Verification items for the finished model (mm, model axes). A direction names the side the tool comes from. Give positions to 0.01 mm unless a question says otherwise; leave off trailing zeros. Loops run counter-clockwise (first coordinate to the right, second up) from the corner with the lowest first, then second, coordinate; pieces in that order, holes last. Notation, with made-up numbers: M 47.5,-37 L 79.5,-37 A21 cw 79.5,-26 Z; hole C 21.5,76.25 d5. An arc over 180 degrees is marked long. Write each question's results on one line, items separated by ' | '. Start each with the question number.
```python
from build123d import *

# Parameters (mm, degrees)
FRAME_BODY_DEPTH         = 40
FRAME_WINDOW_CUT_DEPTH   = 40
SIDE_LUG_A_DEPTH         = 13
SPIGOT_A_SKETCH_R        = 15
SPIGOT_A_SKETCH_R_2      = 7.5
SPIGOT_A_30_DEPTH        = 25
SIDE_START               = 13
SIDE_LUG_B_DEPTH         = 13
SPIGOT_START             = 25
SPIGOT_B_SKETCH_R        = 15
SPIGOT_B_SKETCH_R_2      = 7.5
SPIGOT_B_30_DEPTH        = 25
SPIGOT_EDGE_FILLETS_R2_R = 2
LUG_BLEND_FILLETS_R1_R   = 1


with BuildPart() as part:
    # Frame Profile Sketch → Frame Body (new body)
    with BuildSketch(Plane.XY):
        with BuildLine():
            Line((-12, -64), (12, -64))
            ThreePointArc((12, -64), (21.899494937, -59.899494937), (26, -50))
            Line((26, -50), (26, 50))
            ThreePointArc((26, 50), (21.899494937, 59.899494937), (12, 64))
            Line((12, 64), (-12, 64))
            ThreePointArc((-12, 64), (-21.899494937, 59.899494937), (-26, 50))
            Line((-26, 50), (-26, -50))
            ThreePointArc((-26, -50), (-21.899494937, -59.899494937), (-12, -64))
        make_face()
    extrude(amount=FRAME_BODY_DEPTH)

    # Frame Window Sketch → Frame Window Cut (cut)
    with BuildSketch(Plane.XY.offset(40)):
        with BuildLine():
            Line((14, -35), (14, 35))
            ThreePointArc((14, 35), (18.242640687, 36.757359313), (20, 41))
            Line((20, 41), (20, 50))
            ThreePointArc((20, 50), (18.242640687, 54.242640687), (14, 56))
            Line((14, 56), (-14, 56))
            ThreePointArc((-14, 56), (-18.242640687, 54.242640687), (-20, 50))
            Line((-20, 50), (-20, 41))
            ThreePointArc((-20, 41), (-18.242640687, 36.757359313), (-14, 35))
            Line((-14, 35), (-14, -35))
            ThreePointArc((-14, -35), (-18.242640687, -36.757359313), (-20, -41))
            Line((-20, -41), (-20, -50))
            ThreePointArc((-20, -50), (-18.242640687, -54.242640687), (-14, -56))
            Line((-14, -56), (14, -56))
            ThreePointArc((14, -56), (18.242640687, -54.242640687), (20, -50))
            Line((20, -50), (20, -41))
            ThreePointArc((20, -41), (18.242640687, -36.757359313), (14, -35))
        make_face()
    extrude(amount=-FRAME_WINDOW_CUT_DEPTH, mode=Mode.SUBTRACT)

    # Side Lug A Sketch → Side Lug A (add)
    with BuildSketch(Plane(origin=(26, 0, 0), x_dir=(0, 0, -1), z_dir=(1, 0, 0))):
        with BuildLine():
            Line((-40, 15), (-40, -15))
            ThreePointArc((-40, -15), (-37.914229564, -17.437900652), (-35.533410394, -19.588597743))
            ThreePointArc((-35.533410394, -19.588597743), (-29.708548536, -15.576576016), (-22.978505654, -17.751859172))
            ThreePointArc((-22.978505654, -17.751859172), (-20, -18), (-17.021494346, -17.751859172))
            ThreePointArc((-17.021494346, -17.751859172), (-10.291451464, -15.576576016), (-4.466589606, -19.588597743))
            ThreePointArc((-4.466589606, -19.588597743), (-2.085770436, -17.437900652), (0, -15))
            Line((0, -15), (0, 15))
            ThreePointArc((0, 15), (-2.085770436, 17.437900652), (-4.466589606, 19.588597743))
            ThreePointArc((-4.466589606, 19.588597743), (-10.291451464, 15.576576016), (-17.021494346, 17.751859172))
            ThreePointArc((-17.021494346, 17.751859172), (-20, 18), (-22.978505654, 17.751859172))
            ThreePointArc((-22.978505654, 17.751859172), (-29.708548536, 15.576576016), (-35.533410394, 19.588597743))
            ThreePointArc((-35.533410394, 19.588597743), (-37.914229564, 17.437900652), (-40, 15))
        make_face()
    extrude(amount=SIDE_LUG_A_DEPTH)

    # Spigot A Sketch → Spigot A Ø30 (add)
    with BuildSketch(Plane(origin=(39, 0, 0), x_dir=(0, 0, -1), z_dir=(1, 0, 0))):
        with Locations((-20, 0)):
            Circle(SPIGOT_A_SKETCH_R)
        with Locations((-20, 0)):
            Circle(SPIGOT_A_SKETCH_R_2, mode=Mode.SUBTRACT)
    extrude(amount=SPIGOT_A_30_DEPTH)

    # Side Lug B Sketch → Side Lug B (add)
    with BuildSketch(Plane.ZY.offset(26).offset(SIDE_START)):
        with BuildLine():
            Line((0, 15), (0, -15))
            ThreePointArc((0, -15), (2.085770436, -17.437900652), (4.466589606, -19.588597743))
            ThreePointArc((4.466589606, -19.588597743), (10.291451464, -15.576576016), (17.021494346, -17.751859172))
            ThreePointArc((17.021494346, -17.751859172), (20, -18), (22.978505654, -17.751859172))
            ThreePointArc((22.978505654, -17.751859172), (29.708548536, -15.576576016), (35.533410394, -19.588597743))
            ThreePointArc((35.533410394, -19.588597743), (37.914229564, -17.437900652), (40, -15))
            Line((40, -15), (40, 15))
            ThreePointArc((40, 15), (37.914229564, 17.437900652), (35.533410394, 19.588597743))
            ThreePointArc((35.533410394, 19.588597743), (29.708548536, 15.576576016), (22.978505654, 17.751859172))
            ThreePointArc((22.978505654, 17.751859172), (20, 18), (17.021494346, 17.751859172))
            ThreePointArc((17.021494346, 17.751859172), (10.291451464, 15.576576016), (4.466589606, 19.588597743))
            ThreePointArc((4.466589606, 19.588597743), (2.085770436, 17.437900652), (0, 15))
        make_face()
    extrude(amount=-SIDE_LUG_B_DEPTH)

    # Spigot B Sketch → Spigot B Ø30 (add)
    with BuildSketch(Plane.ZY.offset(39).offset(SPIGOT_START)):
        with Locations(Location((20, 0, 0), (0, 0, 180))):
            Circle(SPIGOT_B_SKETCH_R)
        with Locations(Location((20, 0, 0), (0, 0, 180))):
            Circle(SPIGOT_B_SKETCH_R_2, mode=Mode.SUBTRACT)
    extrude(amount=-SPIGOT_B_30_DEPTH)

    # Spigot Edge Fillets R2
    spigot_edge_fillets_r2_edges = [part.edges().sort_by_distance(p)[0] for p in [
        (64, 0, 35),
        (-64, 0, 35),
    ]]
    fillet(spigot_edge_fillets_r2_edges, radius=SPIGOT_EDGE_FILLETS_R2_R)

    # Lug Blend Fillets R1
    lug_blend_fillets_r1_edges = [part.edges().sort_by_distance(p)[0] for p in [
        (39, 0, 35),
        (-39, 0, 35),
    ]]
    fillet(lug_blend_fillets_r1_edges, radius=LUG_BLEND_FILLETS_R1_R)


solid = part.part
```
1. Thickness scan on probe 1 along X at (y, z) = (-19.5, 7); probe 2 along X at (y, z) = (1.5, 9); probe 3 along Y at (x, z) = (-1.5, 30.5). Record the ranges inside material, lowest first.
2. Section check B-B, the plane y = -21.5. Record the boundary of the cut face in (x, z).
3. Release check for a two-part mould opening along Y. For faces 1 (the face through (26, -33, 20)), 2 (the face through (-32.591, 17.47, 2.117)), 3 (the face through (-18.289, 36.804, 20.28)) record: released by +Y, released by -Y, zero draft, split by the parting line, or undercut.
4. Section check A-A, the plane x = 5. Record the boundary of the cut face in (y, z), plus the area to 3 significant figures.
5. Set-up check for faces 4 (the face through (51.325, 0.33, 27.493)), 5 (the face through (32, 18, 20)), 6 (the face through (32.409, 17.47, 37.883)): record each of +Z, -Z, +X, -X, +Y, -Y from which the full face is reachable in a straight line by a thin tool's end or side.
6. Depth check by flat-ended pin: pin 1 Ø6 at (x, z) = (44, 33.5) entering from -Y; pin 2 Ø10.5 at (y, z) = (-28, 26) entering from +X; pin 3 Ø1 at (y, z) = (-3, 21) entering from -X. Enter the tip coordinate at first touch or a pass-through.
7. Section check C-C, the plane x = -31. Record the boundary of the cut face in (y, z), plus the area to 3 significant figures.
Filled sheet:
1) probe 1: -26 to -14, 14 to 26 | probe 2: -64 to -14, 14 to 64 | probe 3: -64 to -56, 56 to 64
2) outline: M -26,0 L -14,0 L -14,40 L -26,40 Z; M 14,0 L 26,0 L 26,40 L 14,40 Z
3) face 1: zero draft | face 2: released by +Y | face 3: undercut
4) outline: M -64,0 L -56,0 L -56,40 L -64,40 Z; M 56,0 L 64,0 L 64,40 L 56,40 Z | area: 640 mm2
5) face 4: +X | face 5: +X, +Y | face 6: +Z, +X, +Y
6) pin 1: y = -10.71 | pin 2: x = 26 | pin 3: x = -39
7) outline: M -19.59,4.47 A25 ccw -15,0 L 15,0 A25 ccw 19.59,4.47 A8 cw 17.75,17.02 A18 ccw 17.75,22.98 A8 cw 19.59,35.53 A25 ccw 15,40 L -15,40 A25 ccw -19.59,35.53 A8 cw -17.75,22.98 A18 ccw -17.75,17.02 A8 cw Z | area: 1,350 mm2
